Build history of the part. All positions in model axes, mm. A direction names the side the tool comes from. Round coordinates to 2 decimals unless told otherwise and drop trailing zeros. Loops run counter-clockwise (first coordinate to the right, second up) from the corner with the lowest first, then second, coordinate; pieces in that order, holes last.
from build123d import *

# Parameters (mm, degrees)
SKETCH1_W           = 25
SKETCH1_H           = 50
BOSS_EXTRUDE1_DEPTH = 6
SKETCH2_W           = 25
SKETCH2_H           = 20
BOSS_EXTRUDE2_DEPTH = 40
FILLET1_RADIUS      = 12.5
FILLET1_LENGTH      = 6
FILLET3_RADIUS      = 10
FILLET3_LENGTH      = 25
CUT_EXTRUDE1_START  = -5
SKETCH3_W           = 21.31771447
SKETCH3_H           = 40.676557725
CUT_EXTRUDE1_DEPTH  = 15
SKETCH4_R           = 4
CUT_EXTRUDE2_DEPTH  = 59.017238817
SKETCH5_R           = 4.25
CUT_EXTRUDE3_DEPTH  = 49.79805324


with BuildPart() as part:
    # Sketch1 → Boss-Extrude1 (new body)
    with BuildSketch(Plane(origin=(0, 0, 0), x_dir=(1, 0, 0), z_dir=(0, 1, 0))):
        Rectangle(SKETCH1_W, SKETCH1_H)
    extrude(amount=BOSS_EXTRUDE1_DEPTH)

    # Sketch2 → Boss-Extrude2 (add)
    with BuildSketch(Plane(origin=(0, 6, 0), x_dir=(1, 0, 0), z_dir=(0, 1, 0))):
        with Locations((0, -15)):
            Rectangle(SKETCH2_W, SKETCH2_H)
    extrude(amount=BOSS_EXTRUDE2_DEPTH)

    # Fillet1: full round fillet: the end face becomes a half cylinder, R = half its width
    fillet1_face = Plane((0, 3, -25), x_dir=(0, 1, 0), z_dir=(0, 0, -1))  # on the end face: x along it, z out of the body
    fillet1_slab = fillet1_face.offset(-FILLET1_RADIUS / 2) * Box(FILLET1_LENGTH, 2 * FILLET1_RADIUS, FILLET1_RADIUS, mode=Mode.PRIVATE)  # the body's end, R deep
    fillet1_round = Plane((0, 3, -12.5), x_dir=(0, 0, -1), z_dir=(0, 1, 0)) * Cylinder(FILLET1_RADIUS, FILLET1_LENGTH, mode=Mode.PRIVATE)  # its axis R under the face
    add(fillet1_slab - fillet1_round, mode=Mode.SUBTRACT)

    # Fillet3: full round fillet: the end face becomes a half cylinder, R = half its width
    fillet3_face = Plane((0, 46, 15), x_dir=(-1, 0, 0), z_dir=(0, 1, 0))  # on the end face: x along it, z out of the body
    fillet3_slab = fillet3_face.offset(-FILLET3_RADIUS / 2) * Box(FILLET3_LENGTH, 2 * FILLET3_RADIUS, FILLET3_RADIUS, mode=Mode.PRIVATE)  # the body's end, R deep
    fillet3_round = Plane((0, 36, 15), x_dir=(0, 1, 0), z_dir=(-1, 0, 0)) * Cylinder(FILLET3_RADIUS, FILLET3_LENGTH, mode=Mode.PRIVATE)  # its axis R under the face
    add(fillet3_slab - fillet3_round, mode=Mode.SUBTRACT)

    # Sketch3 → Cut-Extrude1 (cut)
    with BuildSketch(Plane.ZY.offset(12.5).offset(CUT_EXTRUDE1_START)):
        with Locations((15.658857235, 39.391263894)):
            Rectangle(SKETCH3_W, SKETCH3_H)
    extrude(amount=-CUT_EXTRUDE1_DEPTH, mode=Mode.SUBTRACT)

    # Sketch4 → Cut-Extrude2 (cut, through all)
    with BuildSketch(Plane.ZY.offset(12.5)):
        with Locations((15, 36)):
            Circle(SKETCH4_R)
    extrude(amount=-CUT_EXTRUDE2_DEPTH, mode=Mode.SUBTRACT)

    # Sketch5 → Cut-Extrude3 (cut, through all)
    with BuildSketch(Plane(origin=(0, 6, 0), x_dir=(1, 0, 0), z_dir=(0, 1, 0))):
        with Locations(Location((0, 7.814758418, 0), (0, 0, 270))):
            Circle(SKETCH5_R)
    extrude(amount=-CUT_EXTRUDE3_DEPTH, mode=Mode.SUBTRACT)


solid = part.part
(1) Probe line 1 (Y direction, x = 10.8, z = 15); line 2 (X direction, y = 22.5, z = 9.5); line 3 (Y direction, x = 10, z = 11.5). List the from-to ranges inside material, lowest first.
Responses:
line 1: y = 0 to 32, 40 to 46
line 2: x = -12.5 to -7.5, 7.5 to 12.5
line 3: y = 0 to 34.06, 37.94 to 45.37
(2) Slice it at A-A on y = 21.5. List the corners of the cut face in (x, z).
Responses:
outline: (-12.5, 5) - (-7.5, 5) - (-7.5, 25) - (-12.5, 25) - close; (7.5, 5) - (12.5, 5) - (12.5, 25) - (7.5, 25) - close
(3) Slice it at C-C on z = 15. List the corners of the cut face in (x, y), plus the area to 3 significant figures.
Responses:
outline: (-12.5, 0) - (12.5, 0) - (12.5, 32) - (7.5, 32) - (7.5, 19.05) - (-7.5, 19.05) - (-7.5, 32) - (-12.5, 32) - close; (-12.5, 40) - (-7.5, 40) - (-7.5, 46) - (-12.5, 46) - close; (7.5, 40) - (12.5, 40) - (12.5, 46) - (7.5, 46) - close
area: 666 mm2
(4) Pin check, flat tips, straight feed: P1, Ø9, axis at y = 36, z = 15, coming from the +X side; P2, Ø1, axis at x = -1, y = 12.5, coming from the -Z side; P3, Ø1.5, axis at x = -5, z = -4.5, coming from the +Y side. Stop position of each tip, or through.
Responses:
P1: stops at x = 12.5
P2: stops at z = 5
P3: stops at y = 6
(5) Slice it at B-B on x = 0. List the corners of the cut face in (y, z), plus the area to 3 significant figures.
Responses:
outline: (0, -25) - (6, -25) - (6, -12.06) - (0, -12.06) - close; (0, -3.56) - (6, -3.56) - (6, 5) - (19.05, 5) - (19.05, 25) - (0, 25) - close
area: 510 mm2
(6) Pull direction Z, two halves, no side cores. Call faces 1 (the face through (2.87, 3.04, -10.95)), 2 (the face through (0, 17, 5)), 3 (the face through (12.5, 18, 15)): +Z half, -Z half, draft (parallel to the pull), parting line (faces both ways), or undercut.
Responses:
face 1: undercut
face 2: -Z half
face 3: draft
(7) Which spindle directions (+Z, -Z, +X, -X, +Y, -Y) get a long thin tool onto all of the face, cutting with end or side? Do faces 4 (the face through (-7.5, 30, 15)), 5 (the face through (0, 6, -14)), 6 (the face through (9.965, 39.966, 14.479)). Say none if no direction does.
Responses:
face 4: +Z, -Z, +Y
face 5: -Z, +X, -X, +Y
face 6: +X, -X
(8) Slice it at D-D on y = 3. List the corners of the cut face in (x, z), plus the area to 3 significant figures.
Responses:
outline: (-12.5, -12.5) arc R12.5 ccw to (12.5, -12.5) - (12.5, 25) - (-12.5, 25) - close; hole circle Ø8.5 at (0, -7.81)
area: 1,130 mm2
